Read the model definition and answer for the solid it produces. Units are mm, in the model's axes. A direction names the side the tool comes from. Give positions to 0.01 mm unless a question says otherwise; leave off trailing zeros. Loops run counter-clockwise (first coordinate to the right, second up) from the corner with the lowest first, then second, coordinate; pieces in that order, holes last. Notation, with made-up numbers: (59.5, 80) - (89.5, 80) arc R36 cw to (89.5, 117) - close; hole circle Ø11 at (9, 38.25). An arc over 180 degrees is marked (long way). Use a Markdown table: item, result. Add a question column.
Item 1: A cutting plane is placed at A-A (x = -50). Determine the outline of the cut face in (y, z), plus the area to 3 significant figures.
Item 2: This flat-tipped pin is pushed along its axis until it touches: P1, Ø10, axis at x = -36, y = 34.5, coming from the +Z side. Where does it stop, or does it pass through?
Item 3: For a pull along Y with two mould halves and no side action, classify faces 1 (the face through (-21, 40, 0)), 2 (the face through (-4, 4, 35)), 3 (the face through (-20, 32, 35)), 4 (the face through (-4, 60, 35)) as +Y half, -Y half, draft (parallel to the pull), parting line (faces both ways), or undercut.
Item 4: Which of the six approach directions +Z, -Z, +X, -X, +Y, -Y give full straight-line access (tool end or side, diameter ignored) to faces 5 (the face through (-42, 21, 35)), 6 (the face through (-50, 4, 35))?
Item 5: Consider probe 1 along Y at (x, z) = (-31, 65); probe 2 along Y at (x, z) = (-29, 51); probe 3 along X at (y, z) = (31.5, 66). Determine where each line is inside the solid, lowest interval first. Write a range as [from, to].
Item 6: A cutting plane is placed at B-B (z = 48). Determine the outline of the cut face in (x, y), plus the area to 3 significant figures.
Item 7: A cutting plane is placed at D-D (x = -25). Determine the outline of the cut face in (y, z), plus the area to 3 significant figures.
Item 8: A cutting plane is placed at C-C (y = 32). Determine the outline of the cut face in (x, z), plus the area to 3 significant figures.
from build123d import *

# Parameters (mm, degrees)
BOSS_EXTRUDE1_DEPTH = 70


with BuildPart() as part:
    # Sketch1 → Boss-Extrude1 (new body)
    with BuildSketch(Plane.XY):
        with BuildLine():
            Line((0, 8), (0, 56))
            Line((0, 56), (-8, 64))
            Line((-8, 64), (-46, 64))
            Line((-46, 64), (-54, 56))
            Line((-54, 56), (-54, 43))
            Line((-54, 43), (-31, 43))
            ThreePointArc((-31, 43), (-20, 32), (-31, 21))
            Line((-31, 21), (-54, 21))
            Line((-54, 21), (-54, 8))
            Line((-54, 8), (-46, 0))
            Line((-46, 0), (-8, 0))
            Line((-8, 0), (0, 8))
        make_face()
    extrude(amount=BOSS_EXTRUDE1_DEPTH)


solid = part.part
Geometry says:
| question | item | result |
|---|---|---|
| 1 | outline | (4, 0) - (21, 0) - (21, 70) - (4, 70) - close; (43, 0) - (60, 0) - (60, 70) - (43, 70) - close |
| 1 | area | 2,380 mm² |
| 2 | P1 | through |
| 3 | face 1 | draft |
| 3 | face 2 | -Y half |
| 3 | face 3 | undercut |
| 3 | face 4 | +Y half |
| 4 | face 5 | +Z, -Z, -X |
| 4 | face 6 | +Z, -Z, -X, -Y |
| 5 | probe 1 | [0, 21], [43, 64] |
| 5 | probe 2 | [0, 21.18], [42.82, 64] |
| 5 | probe 3 | [-20.01, 0] |
| 6 | outline | (-54, 8) - (-46, 0) - (-8, 0) - (0, 8) - (0, 56) - (-8, 64) - (-46, 64) - (-54, 56) - (-54, 43) - (-31, 43) arc R11 cw to (-31, 21) - (-54, 21) - close |
| 6 | area | 2,630 mm² |
| 7 | outline | (0, 0) - (22.78, 0) - (22.78, 70) - (0, 70) - close; (41.22, 0) - (64, 0) - (64, 70) - (41.22, 70) - close |
| 7 | area | 3,190 mm² |
| 8 | outline | (-20, 0) - (0, 0) - (0, 70) - (-20, 70) - close |
| 8 | area | 1,400 mm² |
